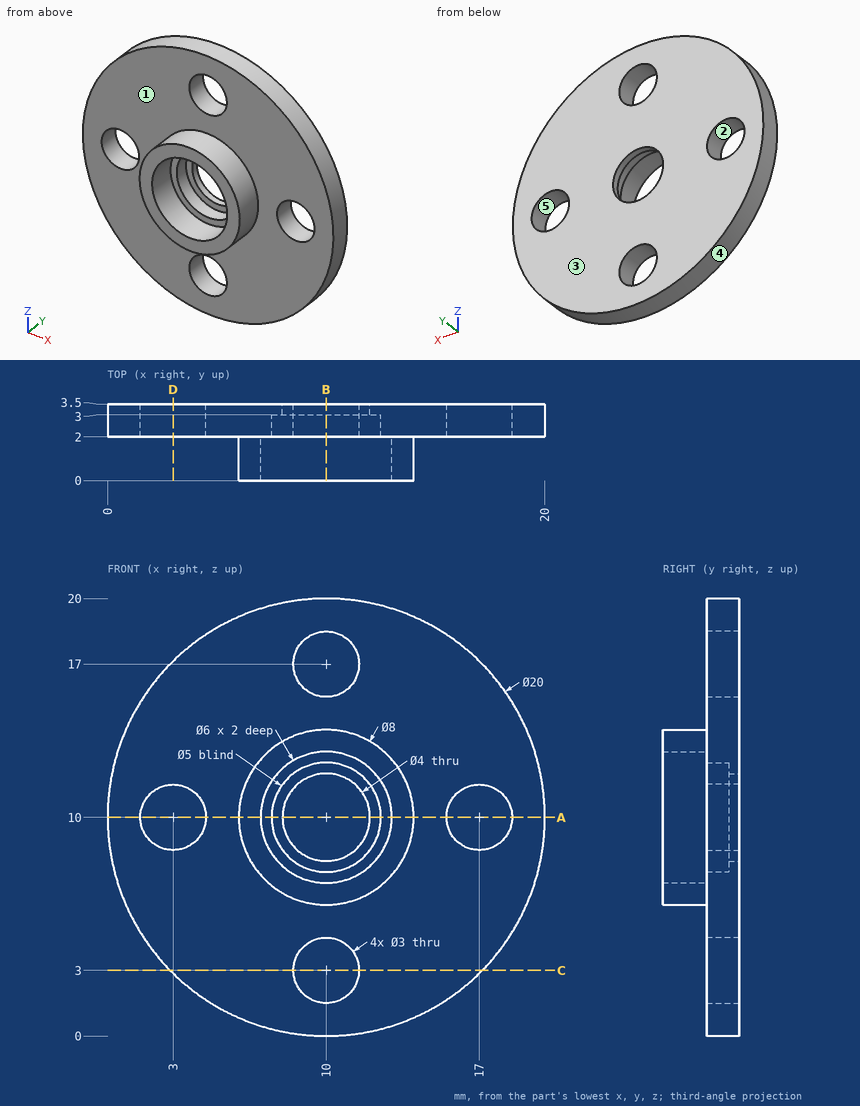
The drawing under review shows one solid part. Ordinate dimensions are in mm from its lowest x, y, z. A direction names the side the tool comes from. Round coordinates to 2 decimals unless told otherwise and drop trailing zeros. Loops run counter-clockwise (first coordinate to the right, second up) from the corner with the lowest first, then second, coordinate; pieces in that order, holes last. Notation, with made-up numbers: (54.25, 56) - (102.25, 56) arc R16 cw to (102.25, 61) - close; hole circle Ø6 at (26, 47). An arc over 180 degrees is marked (long way). Put each result on its own line as item: value. Start each with the question number.
1. Consider section C-C on z = 3. State the section outline as (x, y) points.
2. Mouldability with a two-part tool opening along Z and no side actions: class the marked faces 3, 4 and 5 as +Z half, -Z half, draft (parallel to the pull), parting line (faces both ways), or undercut.
3. For the marked faces 1 and 2, list the 3-axis set-ups (+Z, -Z, +X, -X, +Y, -Y) from which the entire face can be reached by the end or side of a thin tool; tool diameter is ignored.
4. Insertion check: P1, Ø5, axis at x = 17, z = 10, coming from the -Y side; P2, Ø1.5, axis at x = 3, y = 3, coming from the -Z side; P3, Ø2, axis at x = 13.5, y = 1.5, coming from the +Z side. Each pin has a flat end and moves straight along its axis. Give the tip position at first contact, or say it passes through.
5. Consider section A-A on z = 10. State the section outline as (x, y) points, plus the area to 3 significant figures.
6. For probe 1 along X at (y, z) = (2.5, 10); probe 2 along X at (y, z) = (2.65, 11); probe 3 along X at (y, z) = (0.95, 10), list the stretches that pass through material, from the lowest coordinate up. Write a range as [from, to].
7. Consider section D-D on x = 3. State the section outline as (y, z) points.
8. Consider section B-B on x = 10. State the section outline as (y, z) points.
Result sheet:
1. outline: (2.86, 2) - (8.5, 2) - (8.5, 3.5) - (2.86, 3.5) - close; (11.5, 2) - (17.14, 2) - (17.14, 3.5) - (11.5, 3.5) - close
2. face 3: draft
2. face 4: parting line
2. face 5: undercut
3. face 1: -Y
3. face 2: +Y, -Y
4. P1: y = 2
4. P2: z = 2.19
4. P3: z = 19.65
5. outline: (0, 2) - (1.5, 2) - (1.5, 3.5) - (0, 3.5) - close; (4.5, 2) - (6, 2) - (6, 0) - (7, 0) - (7, 2) - (7.5, 2) - (7.5, 3) - (8, 3) - (8, 3.5) - (4.5, 3.5) - close; (12, 3) - (12.5, 3) - (12.5, 2) - (13, 2) - (13, 0) - (14, 0) - (14, 2) - (15.5, 2) - (15.5, 3.5) - (12, 3.5) - close; (18.5, 2) - (20, 2) - (20, 3.5) - (18.5, 3.5) - close
5. area: 18.0 mm^2
6. probe 1: [0, 1.5], [4.5, 7.5], [12.5, 15.5], [18.5, 20]
6. probe 2: [0.05, 1.88], [4.12, 7.71], [12.29, 15.88], [18.12, 19.95]
6. probe 3: [6, 7], [13, 14]
7. outline: (2, 2.86) - (3.5, 2.86) - (3.5, 8.5) - (2, 8.5) - close; (2, 11.5) - (3.5, 11.5) - (3.5, 17.14) - (2, 17.14) - close
8. outline: (0, 6) - (2, 6) - (2, 4.5) - (3.5, 4.5) - (3.5, 8) - (3, 8) - (3, 7.5) - (2, 7.5) - (2, 7) - (0, 7) - close; (0, 13) - (2, 13) - (2, 12.5) - (3, 12.5) - (3, 12) - (3.5, 12) - (3.5, 15.5) - (2, 15.5) - (2, 14) - (0, 14) - close; (2, 0) - (3.5, 0) - (3.5, 1.5) - (2, 1.5) - close; (2, 18.5) - (3.5, 18.5) - (3.5, 20) - (2, 20) - close
